The model under review builds one solid part; all positions refer to its coordinate system, in mm. A direction names the side the tool comes from. Round coordinates to 2 decimals unless told otherwise and drop trailing zeros. Order: outer loops, then holes, each group sorted by start corner. A loop starts at its lowest first (then second) coordinate and runs counter-clockwise, first axis right, second up. Notation, with made-up numbers: M 65.5,49 L 119.5,49 A20 cw 119.5,86 Z; hole C 6,10.5 d11. An arc over 180 degrees is marked long. Answer as a JSON object with one key per item and string values. Group by question number.
1. Clearance check with flat-ended pins moving along their axes: P1, Ø3.5, axis at y = -7, z = -3.5, coming from the -X side; P2, Ø5, axis at x = 91, z = 4.5, coming from the +Y side; P3, Ø5.5, axis at y = -3, z = 1.5, coming from the -X side; P4, Ø6, axis at x = 8.5, z = -1.5, coming from the -Y side. State where each tip first meets the part, or that it passes through.
2. Machinability: for faces 5 (the face through (90, -10, -6.5)), 6 (the face through (19, -5, 0)), 7 (the face through (40, -3, 0)), which of the approach directions +Z, -Z, +X, -X, +Y, -Y give a long, thin tool a straight path to every point of the face, cutting with its end or side? Answer none if there is none.
3. Add section A-A on x = 92. State the section outline as (y, z) points, and give its area (3 significant figures).
4. Add section D-D on x = 15. State the section outline as (y, z) points.
5. Add section C-C on y = -6.75. State the section outline as (x, z) points.
6. Add section B-B on z = 0. State the section outline as (x, y) points.
7. Mouldability with a two-part tool opening along X and no side actions: class faces 1 (the face through (15.06, -2.46, 6.75)), 2 (the face through (31, -13, 0)), 3 (the face through (139, -10, -8)), 4 (the face through (14.94, -2.46, -6.75)) as released by +X, released by -X, zero draft, split by the parting line, or undercut.
8. To check wall thickness, follow probe 1 along Z at (x, y) = (116, -11.25); probe 2 along X at (y, z) = (-1.75, 3); probe 3 along Y at (x, z) = (93.5, 9). State the ranges of each line that lie inside material, in increasing order. Write a range as [from, to].
```python
from build123d import *

# Parameters (mm, degrees)
EXTRUDE_1_DEPTH     = 10
CUT_EXTRUDE_1_DEPTH = 142.155942135
CUT_EXTRUDE_2_DEPTH = 142.155942135
CHAMFER_1_SIZE      = 3
CHAMFER_2_SIZE      = 3
SKETCH_5_W          = 100
SKETCH_5_H          = 5
CUT_EXTRUDE_3_DEPTH = 143.214626533


with BuildPart() as part:
    # 草图2 → 凸台-拉伸1 (new, symmetric)
    with BuildSketch(Plane.XY):
        Polygon((0, 0), (140, 0), (140, -15), (30, -15), (30, -5), (0, -5), align=None)
    extrude(amount=EXTRUDE_1_DEPTH, both=True)

    # 草图3 → 切除-拉伸1 (cut, through all)
    with BuildSketch(Plane(origin=(0, 0, 0), x_dir=(1, 0, 0), z_dir=(0, 1, 0))):
        with BuildLine():
            Line((55, 6.5), (125, 6.5))
            ThreePointArc((125, 6.5), (131.5, 0), (125, -6.5))
            Line((125, -6.5), (55, -6.5))
            ThreePointArc((55, -6.5), (48.5, 0), (55, 6.5))
        make_face()
    extrude(amount=-CUT_EXTRUDE_1_DEPTH, mode=Mode.SUBTRACT)

    # 草图4 → 切除-拉伸2 (cut, through all)
    with BuildSketch(Plane(origin=(0, 0, 0), x_dir=(1, 0, 0), z_dir=(0, 1, 0))):
        with BuildLine():
            Line((17.75, 4), (17.75, -4))
            ThreePointArc((17.75, -4), (15, -6.75), (12.25, -4))
            Line((12.25, -4), (12.25, 4))
            ThreePointArc((12.25, 4), (15, 6.75), (17.75, 4))
        make_face()
    extrude(amount=-CUT_EXTRUDE_2_DEPTH, mode=Mode.SUBTRACT)

    # 倒角1
    chamfer_1_edges = [part.edges().sort_by_distance(p)[0] for p in [
        (140, -7.5, 10),
        (140, -7.5, -10),
    ]]
    chamfer(chamfer_1_edges, length=CHAMFER_1_SIZE)

    # 倒角2
    chamfer_2_edges = [part.edges().sort_by_distance(p)[0] for p in [
        (30, -15, 0),
    ]]
    chamfer(chamfer_2_edges, length=CHAMFER_2_SIZE)

    # 草图5 → 切除-拉伸3 (cut, through all)
    with BuildSketch(Plane.XY.offset(10)):
        with Locations((90, -2.5)):
            Rectangle(SKETCH_5_W, SKETCH_5_H)
    extrude(amount=-CUT_EXTRUDE_3_DEPTH, mode=Mode.SUBTRACT)


solid = part.part
```
Recorded:
{
 "1": {"P1": "stops at x = 30", "P2": "stops at y = -5", "P3": "stops at x = 0", "P4": "stops at y = -5"},
 "2": {"face 5": "+Y, -Y", "face 6": "+Z, -Z, -X, -Y", "face 7": "+Z, -Z, +X, +Y"},
 "3": {"outline": "M -15,-10 L -5,-10 L -5,-6.5 L -15,-6.5 Z; M -15,6.5 L -5,6.5 L -5,10 L -15,10 Z", "area": "70.0 mm²"},
 "4": {"outline": "M -5,-10 L 0,-10 L 0,-6.75 L -5,-6.75 Z; M -5,6.75 L 0,6.75 L 0,10 L -5,10 Z"},
 "5": {"outline": "M 30,-10 L 137,-10 L 140,-7 L 140,7 L 137,10 L 30,10 Z; hole M 55,-6.5 L 125,-6.5 A6.5 ccw 125,6.5 L 55,6.5 A6.5 ccw Z"},
 "6": {"outline": "M 0,-5 L 12.25,-5 L 12.25,0 L 0,0 Z; M 17.75,-5 L 30,-5 L 30,-12 L 33,-15 L 48.5,-15 L 48.5,-5 L 40,-5 L 40,0 L 17.75,0 Z; M 131.5,-15 L 140,-15 L 140,-5 L 131.5,-5 Z"},
 "7": {"face 1": "undercut", "face 2": "released by -X", "face 3": "released by +X", "face 4": "undercut"},
 "8": {"probe 1": "z = [-10, -6.5], [6.5, 10]", "probe 2": "x = [0, 12.25], [17.75, 40]", "probe 3": "y = [-15, -5]"}
}
